Verification items for the finished model (mm, model axes). Face numbers are marked on the shaded views. A direction names the side the tool comes from. Give positions to 0.01 mm unless a question says otherwise; leave off trailing zeros. Write each loop counter-clockwise with the first axis right and the second up, starting at its lowest first coordinate (ties: lowest second). Pieces come first, ordered by that corner, then holes. Notation, with made-up numbers: (-29, 15.5) - (-5, 15.5) arc R26 ccw to (-5, 39.5) - close; hole circle Ø9 at (47.25, 41). An arc over 180 degrees is marked (long way). Put each result on its own line as item: value.
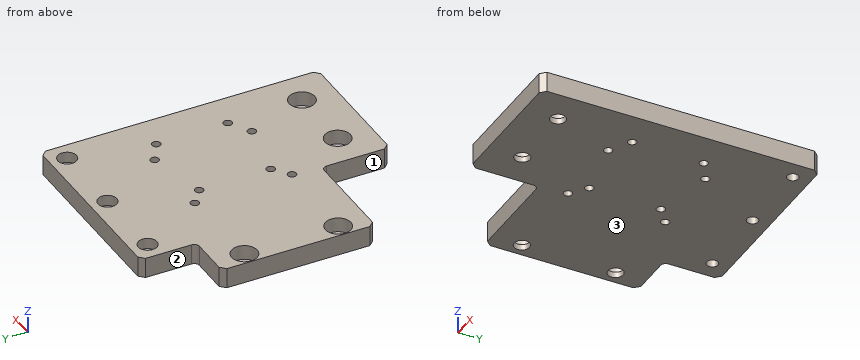
from build123d import *

# Parameters (mm, degrees)
SKETCH_1_W                     = 140
SKETCH_1_H                     = 112
EXTRUDE_1_DEPTH                = 12
HOLE_WIZARD_M6_1_D             = 5
HOLE_WIZARD_M6_2_D             = 5
SKETCH_6_W                     = 112
SKETCH_6_H                     = 12
EXTRUDE_2_DEPTH                = 22
SKETCH_7_W                     = 28
SKETCH_7_H                     = 12
CUT_EXTRUDE_1_DEPTH            = 11
SKETCH_8_W                     = 60
SKETCH_8_H                     = 12
CUT_EXTRUDE_2_DEPTH            = 11
HOLE_WIZARD_M6_1_2_D           = 6.6
HOLE_WIZARD_M6_1_2_CBORE_D     = 11
HOLE_WIZARD_M6_1_2_CBORE_DEPTH = 6.4
SKETCH_11_W                    = 80
SKETCH_11_H                    = 12
EXTRUDE_3_DEPTH                = 29
CHAMFER_1_SIZE                 = 3
FILLET_1_R                     = 3
HOLE_WIZARD_M8_1_D             = 9
HOLE_WIZARD_M8_1_CBORE_D       = 15
HOLE_WIZARD_M8_1_CBORE_DEPTH   = 8.6
HOLE_WIZARD_M8_2_D             = 9
HOLE_WIZARD_M8_2_CBORE_D       = 15
HOLE_WIZARD_M8_2_CBORE_DEPTH   = 8.6


with BuildPart() as part:
    # 草图1 → 凸台-拉伸1 (new body)
    with BuildSketch(Plane.XY):
        with Locations((70, 56)):
            Rectangle(SKETCH_1_W, SKETCH_1_H)
    extrude(amount=EXTRUDE_1_DEPTH)

    # Hole Wizard M6 _1 (through all)
    with Locations(Plane(origin=(0, 0, 0), x_dir=(-1, 0, 0), z_dir=(0, 0, -1))):
        with Locations((-106.5, 84.5), (-61.5, 84.5), (-61.5, 27.5), (-106.5, 27.5)):
            Hole(HOLE_WIZARD_M6_1_D / 2)

    # M6 螺纹孔2 (through all)
    with Locations(Plane.XY.offset(12)):
        with Locations((71, 77), (71, 35), (119, 35), (119, 77)):
            Hole(HOLE_WIZARD_M6_2_D / 2)

    # 草图6 → 凸台-拉伸2 (add)
    with BuildSketch(Plane(origin=(0, 112, 0), x_dir=(1, 0, 0), z_dir=(0, 1, 0))):
        with Locations((84, -6)):
            Rectangle(SKETCH_6_W, SKETCH_6_H)
    extrude(amount=EXTRUDE_2_DEPTH)

    # 草图7 → 切除-拉伸1 (cut)
    with BuildSketch(Plane(origin=(0, 112, 0), x_dir=(1, 0, 0), z_dir=(0, 1, 0))):
        with Locations((14, -6)):
            Rectangle(SKETCH_7_W, SKETCH_7_H)
    extrude(amount=-CUT_EXTRUDE_1_DEPTH, mode=Mode.SUBTRACT)

    # 草图8 → 切除-拉伸2 (cut)
    with BuildSketch(Plane.XZ):
        with Locations((30, 6)):
            Rectangle(SKETCH_8_W, SKETCH_8_H)
    extrude(amount=-CUT_EXTRUDE_2_DEPTH, mode=Mode.SUBTRACT)

    # Hole Wizard M6 _1 2 (through all)
    with Locations(Plane.XY.offset(12)):
        with Locations((129, 124), (84, 124), (39, 124)):
            CounterBoreHole(HOLE_WIZARD_M6_1_2_D / 2, HOLE_WIZARD_M6_1_2_CBORE_D / 2, HOLE_WIZARD_M6_1_2_CBORE_DEPTH)

    # 草图11 → 凸台-拉伸3 (add)
    with BuildSketch(Plane.XZ):
        with Locations((100, 6)):
            Rectangle(SKETCH_11_W, SKETCH_11_H)
    extrude(amount=EXTRUDE_3_DEPTH)

    # 倒角1
    chamfer_1_edges = [part.edges().sort_by_distance(p)[0] for p in [
        (140, -29, 6),
        (60, -29, 6),
        (0, 11, 6),
        (140, 134, 6),
        (0, 101, 6),
        (28, 134, 6),
    ]]
    chamfer(chamfer_1_edges, length=CHAMFER_1_SIZE)

    # 圆角1
    fillet_1_edges = [part.edges().sort_by_distance(p)[0] for p in [
        (28, 101, 6),
        (60, 11, 6),
    ]]
    fillet(fillet_1_edges, radius=FILLET_1_R)

    # M8 六角凹头螺钉的柱形沉头孔1 (through all)
    with Locations(Plane.XY.offset(12)):
        with Locations((8, 83.5), (8, 28.5)):
            CounterBoreHole(HOLE_WIZARD_M8_1_D / 2, HOLE_WIZARD_M8_1_CBORE_D / 2, HOLE_WIZARD_M8_1_CBORE_DEPTH)

    # M8 六角凹头螺钉的柱形沉头孔2 (through all)
    with Locations(Plane.XY.offset(12)):
        with Locations((80, -9), (120, -9)):
            CounterBoreHole(HOLE_WIZARD_M8_2_D / 2, HOLE_WIZARD_M8_2_CBORE_D / 2, HOLE_WIZARD_M8_2_CBORE_DEPTH)


solid = part.part
Q1. Section check D-D, the plane x = 82.5. Record the cut outline in (y, z).
Answers follow:
outline: (-29, 0) - (-12.74, 0) - (-12.74, 3.4) - (-16.07, 3.4) - (-16.07, 12) - (-29, 12) - close; (-5.26, 0) - (121.06, 0) - (121.06, 5.6) - (118.71, 5.6) - (118.71, 12) - (-1.93, 12) - (-1.93, 3.4) - (-5.26, 3.4) - close; (126.94, 0) - (134, 0) - (134, 12) - (129.29, 12) - (129.29, 5.6) - (126.94, 5.6) - close
Q2. Section check A-A, the plane x = 39. Record the cut outline in (y, z), plus the area to 3 significant figures.
Answers follow:
outline: (11, 0) - (120.7, 0) - (120.7, 5.6) - (118.5, 5.6) - (118.5, 12) - (11, 12) - close; (127.3, 0) - (134, 0) - (134, 12) - (129.5, 12) - (129.5, 5.6) - (127.3, 5.6) - close
area: 1,370 mm2
Q3. Go/stop test with flat-tipped pins: pin 1 Ø3.5 at (x, y) = (83.5, 122) entering from +Z; pin 2 Ø6.5 at (x, y) = (106.5, 84.5) entering from -Z; pin 3 Ø4 at (x, y) = (119, 77) entering from +Z; pin 4 Ø6 at (x, z) = (18, 3) entering from -Y. Record where each tip stops, or that it passes through.
Answers follow:
pin 1: stops at z = 5.6
pin 2: stops at z = 0
pin 3: passes through
pin 4: stops at y = 11
Q4. Section check B-B, the plane z = 9.5. Give the number of separate pieces and of enclosed holes in the cut face, plus the area to 3 significant figures.
Answers follow:
separate pieces: 1
enclosed holes: 15
area: 18,300 mm2
Q5. Section check C-C, the plane x = 119. Record the cut outline in (y, z), plus the area to 3 significant figures.
Answers follow:
outline: (-29, 0) - (-13.39, 0) - (-13.39, 3.4) - (-16.43, 3.4) - (-16.43, 12) - (-29, 12) - close; (-4.61, 0) - (32.5, 0) - (32.5, 12) - (-1.57, 12) - (-1.57, 3.4) - (-4.61, 3.4) - close; (37.5, 0) - (74.5, 0) - (74.5, 12) - (37.5, 12) - close; (79.5, 0) - (134, 0) - (134, 12) - (79.5, 12) - close
area: 1,680 mm2
Q6. Set-up check for the marked faces 1, 2 and 3: record each of +Z, -Z, +X, -X, +Y, -Y from which the full face is reachable in a straight line by a thin tool's end or side.
Answers follow:
face 1: +Z, -Z, -X, -Y
face 2: +Z, -Z, -X, +Y
face 3: -Z, +X, -X, +Y, -Y
Q7. Scan lines: line 1 along X through (y, z) = (-8.5, 5); line 2 along Y through (x, z) = (71, 2.75); line 3 along Y through (x, z) = (80, 5.75). Record each from-to range of solid material in increasing order.
Answers follow:
line 1: x = 60 to 72.52, 87.48 to 112.52, 127.48 to 140
line 2: y = -29 to 32.5, 37.5 to 74.5, 79.5 to 134
line 3: y = -29 to -16.5, -1.5 to 120.23, 127.77 to 134
